Read the model definition and answer for the solid it produces. Units are mm, in the model's axes. Face numbers are marked on the shaded views. A direction names the side the tool comes from. Coordinates: 2 decimals unless noted, no trailing zeros. Loops run counter-clockwise (first coordinate to the right, second up) from the corner with the lowest first, then second, coordinate; pieces in that order, holes last. Notation, with made-up numbers: (6, 42.5) -> (11, 42.5) arc R21 ccw to (11, 52.5) -> close; hole circle Ø8 at (-18.75, 73.25). An arc over 180 degrees is marked (long way). Answer in a Markdown table with one row per item.
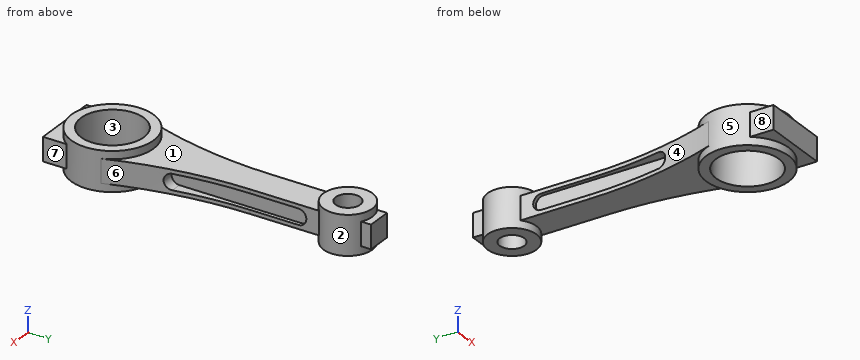
```python
from build123d import *

# Parameters (mm, degrees)
ROD_PROFILE_SKETCH_R   = 12.5
ROD_PROFILE_SKETCH_R_2 = 6.25
ROD_BODY_DEPTH         = 10
ROD_PROFILE_SKETCH_R_3 = 21
ROD_PROFILE_SKETCH_R_4 = 16
ROD_BODY_2_DEPTH       = 10
EYE_BOSS_DEPTH         = 6
WEB_START              = 6
WEB_RECESS_CUT_DEPTH   = 132.802456026


with BuildPart() as part:
    # Rod Profile Sketch → Rod Body (new, symmetric)
    with BuildSketch(Plane.XY):
        with Locations((0, 120)):
            Circle(ROD_PROFILE_SKETCH_R)
        with Locations((0, 120)):
            Circle(ROD_PROFILE_SKETCH_R_2, mode=Mode.SUBTRACT)
    extrude(amount=ROD_BODY_DEPTH, both=True)



with BuildPart() as body_2:
    # Rod Profile Sketch → Rod Body 2 (new, symmetric)
    with BuildSketch(Plane.XY):
        Circle(ROD_PROFILE_SKETCH_R_3)
        Circle(ROD_PROFILE_SKETCH_R_4, mode=Mode.SUBTRACT)
    extrude(amount=ROD_BODY_2_DEPTH, both=True)


with BuildPart() as part_1:
    add(part.part)

    add(body_2.part)  # Eye Boss merges body 2
    # Sketch1_3 → Eye Boss (add, symmetric)
    with BuildSketch(Plane.XY):
        with BuildLine():
            Line((-8, 110.395313644), (-8, 75.395313644))
            ThreePointArc((-8, 75.395313644), (-10.96842855, 40.709642053), (-19.787382488, 7.032744434))
            ThreePointArc((-19.787382488, 7.032744434), (0, 21), (19.787382488, 7.032744434))
            ThreePointArc((19.787382488, 7.032744434), (10.96842855, 40.709642053), (8, 75.395313644))
            Line((8, 75.395313644), (8, 110.395313644))
            ThreePointArc((8, 110.395313644), (0, 107.5), (-8, 110.395313644))
        make_face()
        with BuildLine():
            Line((-6.25, 135.825317547), (-6.25, 130.825317547))
            ThreePointArc((-6.25, 130.825317547), (0, 132.5), (6.25, 130.825317547))
            Line((6.25, 130.825317547), (6.25, 135.825317547))
            Line((6.25, 135.825317547), (-6.25, 135.825317547))
        make_face()
        with BuildLine():
            ThreePointArc((17, -12.328828006), (0, -21), (-17, -12.328828006))
            Line((-17, -12.328828006), (-17, -24.328828006))
            Line((-17, -24.328828006), (17, -24.328828006))
            Line((17, -24.328828006), (17, -12.328828006))
        make_face()
    extrude(amount=EYE_BOSS_DEPTH, both=True)

    # Web Recess Sketch → Web Recess Cut (cut, through all)
    with BuildSketch(Plane(origin=(0, 0, 0), x_dir=(0, 0, -1), z_dir=(1, 0, 0)).offset(WEB_START)):
        with BuildLine():
            Line((4, 100), (4, 38))
            ThreePointArc((4, 38), (0, 34), (-4, 38))
            Line((-4, 38), (-4, 100))
            ThreePointArc((-4, 100), (0, 104), (4, 100))
        make_face()
    web_recess_cut = extrude(amount=WEB_RECESS_CUT_DEPTH, mode=Mode.SUBTRACT)

    # Web Recess Mirror: Web Recess Cut across plane
    add(web_recess_cut.mirror(Plane(origin=(0, 0, 0), x_dir=(0, 0, 1), z_dir=(1, 0, 0))), mode=Mode.SUBTRACT)


solid = part_1.part
```
1. A cutting plane is placed at A-A on y = 120. Give the vertices of the cut face in (x, z), and give its area (3 significant figures).
A:
| item | result |
|---|---|
| outline | (-12.5, -10) -> (-6.25, -10) -> (-6.25, 10) -> (-12.5, 10) -> close; (6.25, -10) -> (12.5, -10) -> (12.5, 10) -> (6.25, 10) -> close |
| area | 250 mm2 |
2. The mould has two halves that part along X. Classify the marked faces 1, 2, 3 and 4: pulls with the +X half, pulls with the -X half, needs draft (parallel to the pull), parting line crosses it, or undercut.
A:
| item | result |
|---|---|
| face 1 | needs draft |
| face 2 | parting line crosses it |
| face 3 | undercut |
| face 4 | pulls with the -X half |
3. A cutting plane is placed at D-D on z = 7.5. Give the vertices of the cut face in (x, y), and give its area (3 significant figures).
A:
| item | result |
|---|---|
| outline | circle Ø42 at (0, 0); circle Ø25 at (0, 120); hole circle Ø32 at (0, 0); hole circle Ø12.5 at (0, 120) |
| area | 949 mm2 |
4. A cutting plane is placed at C-C on x = 0. Give the vertices of the cut face in (y, z).
A:
| item | result |
|---|---|
| outline | (-24.33, -6) -> (-21, -6) -> (-21, -10) -> (-16, -10) -> (-16, 10) -> (-21, 10) -> (-21, 6) -> (-24.33, 6) -> close; (16, -10) -> (21, -10) -> (21, -6) -> (107.5, -6) -> (107.5, -10) -> (113.75, -10) -> (113.75, 10) -> (107.5, 10) -> (107.5, 6) -> (21, 6) -> (21, 10) -> (16, 10) -> close; (126.25, -10) -> (132.5, -10) -> (132.5, -6) -> (135.83, -6) -> (135.83, 6) -> (132.5, 6) -> (132.5, 10) -> (126.25, 10) -> close |
5. Given pin 1 Ø1.5 at (y, z) = (69.5, 0) entering from +X; pin 2 Ø10 at (x, y) = (12, 86.5) entering from -Z; pin 3 Ø6 at (y, z) = (-20.5, -2) entering from -X, each flat-ended and moving along its own axis, determine where each tip first touches the part or whether it passes through.
A:
| item | result |
|---|---|
| pin 1 | stops at x = 6 |
| pin 2 | stops at z = -6 |
| pin 3 | stops at x = -17 |
6. A tool of negligible diameter and unlimited length cuts with its end or side. For the marked faces 5, 6, 7 and 8, from which of +Z, -Z, +X, -X, +Y, -Y can it reach the whole face along a straight path? Write none if from no direction.
A:
| item | result |
|---|---|
| face 5 | none |
| face 6 | +Z, -Z, +X |
| face 7 | +Z, -Z, +X, -Y |
| face 8 | +Z, -Z, -X, -Y |
7. Find the intervals of material crossed by probe 1 along Y at (x, z) = (0, -1.25); probe 2 along Z at (x, y) = (-7.5, 90); probe 3 along Y at (x, z) = (2, -7), in increasing order.
A:
| item | result |
|---|---|
| probe 1 | y = -24.33 to -16, 16 to 113.75, 126.25 to 135.83 |
| probe 2 | z = -6 to -4, 4 to 6 |
| probe 3 | y = -20.9 to -15.87, 15.87 to 20.9, 107.66 to 114.08, 125.92 to 132.34 |
8. A cutting plane is placed at B-B on z = 0. Give the vertices of the cut face in (x, y).
A:
| item | result |
|---|---|
| outline | (-19.79, 7.03) arc R21 ccw to (-17, -12.33) -> (-17, -24.33) -> (17, -24.33) -> (17, -12.33) arc R21 ccw to (19.79, 7.03) arc R204.13 cw to (12.24, 34) -> (6, 34) -> (6, 104) -> (8, 104) -> (8, 110.4) arc R12.5 ccw to (6.25, 130.83) -> (6.25, 135.83) -> (-6.25, 135.83) -> (-6.25, 130.83) arc R12.5 ccw to (-8, 110.4) -> (-8, 104) -> (-6, 104) -> (-6, 34) -> (-12.24, 34) arc R204.13 cw to start; hole circle Ø32 at (0, 0); hole circle Ø12.5 at (0, 120) |
